Verification items for the finished model (mm, model axes). Face numbers are marked on the shaded views. A direction names the side the tool comes from. Round coordinates to 2 decimals unless told otherwise and drop trailing zeros. Write each loop counter-clockwise with the first axis right and the second up, starting at its lowest first coordinate (ties: lowest second). Pieces come first, ordered by that corner, then holes. Notation, with made-up numbers: M 87,31 L 105,31 A21 cw 105,35 Z; hole C -32.75,-15.5 d9. An arc over 180 degrees is marked long. One line per item, written item: value. Start each with the question number.
Item 1: Section check A-A, the plane x = 35. Record the cut outline in (y, z), then the cut area to 4 significant figures.
Item 2: Gauge pin test, flat ends, axial feed: pin 1 (17 mm diameter, centred on x = 109.5, z = -34.5, fed in from -Y); pin 2 (6 mm diameter, centred on y = -38.5, z = -16.5, fed in from +X); pin 3 (12.5 mm diameter, centred on x = 106.5, z = 34.5, fed in from -Y); pin 4 (12 mm diameter, centred on x = 53, y = -53, fed in from +Z). Record the tip position at first contact, or that the pin passes through.
Item 3: Section check D-D, the plane z = 13. Record the cut outline in (x, y).
Item 4: Thickness scan on probe 1 along X at (y, z) = (-32, -35); probe 2 along Y at (x, z) = (64, -33); probe 3 along X at (y, z) = (-16, -35). Record the ranges inside material, lowest first. Write a range as from..to.
Item 5: Section check C-C, the plane x = 172. Record the cut outline in (y, z).
Item 6: Section check B-B, the plane y = -20.5. Record the cut outline in (x, z).
Item 7: Tool access check on the marked faces 5 and 6. Record the directions out of +Z, -Z, +X, -X, +Y, -Y that give a thin tool (end or side, any length) a straight path to the whole face; none if there is none.
Item 8: Draft check along X on the marked faces 1, 2, 3 and 4. Enter one of: +X half, -X half, draft (parallel to the pull), parting line (faces both ways), or undercut.
from build123d import *

# Parameters (mm, degrees)
BASE_BLOCK_SKETCH_W   = 200
BASE_BLOCK_SKETCH_H   = 125
BASE_BLOCK_DEPTH      = 50
UPPER_BLOCK_DEPTH     = 50
LUG_BOSS_DEPTH        = 30
LUG_BORE_SKETCH_R     = 20
LUG_BORE_DEPTH        = 50
CHANNEL_CUT_DEPTH     = 200
CORNER_TRIM_CUT_DEPTH = 200
TAPER_FILL_1_DEPTH    = 80
TAPER_FILL_2_DEPTH    = 80


with BuildPart() as part:
    # Base Block Sketch → Base Block (new body)
    with BuildSketch(Plane.XY):
        with Locations((100, -62.5)):
            Rectangle(BASE_BLOCK_SKETCH_W, BASE_BLOCK_SKETCH_H)
    extrude(amount=BASE_BLOCK_DEPTH)

    # Upper Block Sketch → Upper Block (add)
    with BuildSketch(Plane(origin=(0, 0, 0), x_dir=(1, 0, 0), z_dir=(0, 1, 0))):
        with BuildLine():
            Line((0, 0), (70, 0))
            Line((70, 0), (70, 35))
            ThreePointArc((70, 35), (35, 70), (0, 35))
            Line((0, 35), (0, 0))
        make_face()
    extrude(amount=-UPPER_BLOCK_DEPTH)

    # Lug Sketch → Lug Boss (add)
    with BuildSketch(Plane(origin=(0, 0, 0), x_dir=(1, 0, 0), z_dir=(0, 1, 0))):
        with BuildLine():
            Line((70, 0), (130, 0))
            Line((130, 0), (62.686080753, 56.412167861))
            ThreePointArc((62.686080753, 56.412167861), (68.121087138, 46.31342507), (70, 35))
            Line((70, 35), (70, 0))
        make_face()
    extrude(amount=-LUG_BOSS_DEPTH)

    # Lug Bore Sketch → Lug Bore (cut)
    with BuildSketch(Plane.XZ.offset(50)):
        with Locations(Location((35, -35, 0), (0, 0, 270))):
            Circle(LUG_BORE_SKETCH_R)
    extrude(amount=-LUG_BORE_DEPTH, mode=Mode.SUBTRACT)

    # Channel Sketch → Channel Cut (cut)
    with BuildSketch(Plane(origin=(200, 0, 0), x_dir=(0, 0, -1), z_dir=(1, 0, 0))):
        Polygon((-50, -62.5), (-50, -25), (-25, -25), (-25, -100), (-50, -100), align=None)
    extrude(amount=-CHANNEL_CUT_DEPTH, mode=Mode.SUBTRACT)

    # Corner Trim Sketch → Corner Trim Cut (cut)
    with BuildSketch(Plane(origin=(200, 0, 0), x_dir=(0, 0, -1), z_dir=(1, 0, 0))):
        Polygon((-50, -125), (0.050929029, -106.782951636), (0, -125), align=None)
    extrude(amount=-CORNER_TRIM_CUT_DEPTH, mode=Mode.SUBTRACT)

    # Taper Fill 1 Sketch → Taper Fill 1 (add)
    with BuildSketch(Plane(origin=(200, 0, 0), x_dir=(0, 0, -1), z_dir=(1, 0, 0))):
        Polygon((-50, -125), (0, -106.801488287), (0, -125), align=None)
    extrude(amount=-TAPER_FILL_1_DEPTH)

    # Taper Fill 2 Sketch → Taper Fill 2 (add)
    with BuildSketch(Plane.ZY):
        Polygon((0, -106.801488287), (50, -125), (0, -125), align=None)
    extrude(amount=-TAPER_FILL_2_DEPTH)


solid = part.part
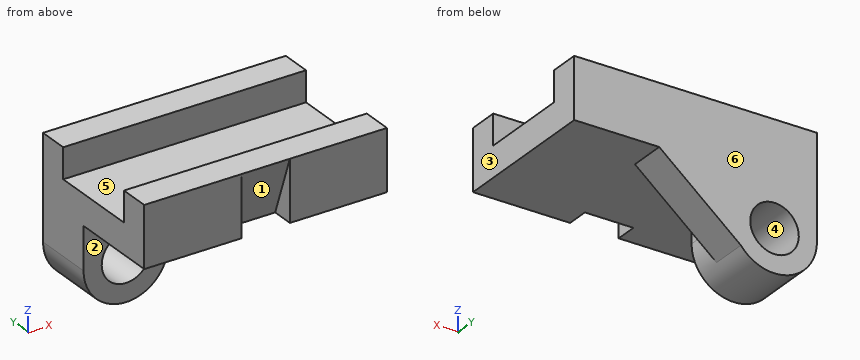
Response values:
1. outline: M -125,0 L -50,0 L -50,-15 L 0,-15 L 0,50 L -25,50 L -25,25 L -100,25 L -100,50 L -125,50 Z; M -50,-70 L 0,-70 L 0,-55 L -50,-55 Z
1. area: 5,875 mm2
2. pin 1: passes through
2. pin 2: stops at x = 70
2. pin 3: stops at y = -121.63
2. pin 4: stops at z = 25
3. outline: M 0,-125 L 80,-125 L 80,-111.53 L 120,-111.53 L 120,-125 L 200,-125 L 200,0 L 0,0 Z
4. probe 1: x = 0..15, 55..70
4. probe 2: y = -50..0
4. probe 3: x = 0..15, 55..88.24
5. outline: M -125,0 L 0,0 L 0,50 L -25,50 L -25,25 L -100,25 L -100,50 L -125,50 Z
6. outline: M 0,-35 A35 ccw 62.69,-56.41 L 130,0 L 200,0 L 200,50 L 0,50 Z; hole C 35,-35 d40
7. face 5: +Z, +X, -X
7. face 6: +Z, -Z, +X, -X, +Y
8. face 1: undercut
8. face 2: draft
8. face 3: +X half
8. face 4: undercut
